Design review of the part built by this model. Coordinates are the model's own, in mm. Face numbers are marked on the shaded views. A direction names the side the tool comes from. Give positions to 0.01 mm unless a question says otherwise; leave off trailing zeros. Loops run counter-clockwise (first coordinate to the right, second up) from the corner with the lowest first, then second, coordinate; pieces in that order, holes last. Notation, with made-up numbers: M 21.5,76.5 L 52.5,76.5 A15 ccw 52.5,99.5 Z; hole C -24,-21.5 d1. An arc over 180 degrees is marked long. Use CSV: the item, a comma, the result in double quotes.
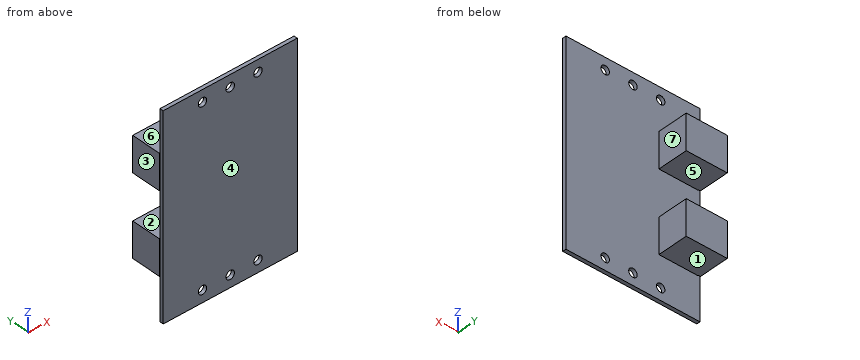
from build123d import *

# Parameters (mm, degrees)
SKETCH_1_W          = 60.4
SKETCH_1_H          = 89.7
EXTRUDE_1_DEPTH     = 1.6
SKETCH_2_R          = 1.9
CUT_EXTRUDE_1_DEPTH = 1.6
SKETCH_3_W          = 15.8
SKETCH_3_H          = 13.7
EXTRUDE_2_DEPTH     = 18.5
SKETCH_4_W          = 51.8
SKETCH_4_H          = 0.2
CUT_EXTRUDE_2_DEPTH = 1


with BuildPart() as part:
    # 草图1 → 凸台-拉伸1 (new body)
    with BuildSketch(Plane(origin=(0, 0, 0), x_dir=(1, 0, 0), z_dir=(0, 1, 0))):
        Rectangle(SKETCH_1_W, SKETCH_1_H)
    extrude(amount=EXTRUDE_1_DEPTH)

    # 草图2 → 切除-拉伸1 (cut)
    with BuildSketch(Plane(origin=(0, 1.6, 0), x_dir=(1, 0, 0), z_dir=(0, 1, 0))):
        with Locations(Location((-12.5, -39.5, 0), (0, 0, 270))):
            Circle(SKETCH_2_R)
        with Locations(Location((12.5, -39.5, 0), (0, 0, 270))):
            Circle(SKETCH_2_R)
        with Locations(Location((-12.5, 39.5, 0), (0, 0, 270))):
            Circle(SKETCH_2_R)
        with Locations(Location((12.5, 39.5, 0), (0, 0, 270))):
            Circle(SKETCH_2_R)
        with Locations(Location((0, 39.5, 0), (0, 0, 270))):
            Circle(SKETCH_2_R)
        with Locations(Location((0, -39.5, 0), (0, 0, 270))):
            Circle(SKETCH_2_R)
    extrude(amount=-CUT_EXTRUDE_1_DEPTH, mode=Mode.SUBTRACT)

    # 草图3 → 凸台-拉伸2 (add)
    with BuildSketch(Plane.ZY.offset(30.2)):
        with Locations((18, 8.45)):
            Rectangle(SKETCH_3_W, SKETCH_3_H)
        with Locations((-18, 8.45)):
            Rectangle(SKETCH_3_W, SKETCH_3_H)
    extrude(amount=-EXTRUDE_2_DEPTH)

    # 草图4 → 切除-拉伸2 (cut)
    with BuildSketch(Plane.ZY.offset(30.2)):
        with Locations((0, 1.7)):
            Rectangle(SKETCH_4_W, SKETCH_4_H)
    extrude(amount=-CUT_EXTRUDE_2_DEPTH, mode=Mode.SUBTRACT)


solid = part.part
(1) We need section D-D on x = -22. State the section outline as (y, z) points, then the cut area to 3 significant figures.
A:
outline,"M 0,-44.85 L 1.6,-44.85 L 1.6,-25.9 L 15.3,-25.9 L 15.3,-10.1 L 1.6,-10.1 L 1.6,10.1 L 15.3,10.1 L 15.3,25.9 L 1.6,25.9 L 1.6,44.85 L 0,44.85 Z"
area,"576 mm²"
(2) We need section A-A on z = -39.5. State the section outline as (x, y) points.
A:
outline,"M -30.2,0 L -14.4,0 L -14.4,1.6 L -30.2,1.6 Z; M -10.6,0 L -1.9,0 L -1.9,1.6 L -10.6,1.6 Z; M 1.9,0 L 10.6,0 L 10.6,1.6 L 1.9,1.6 Z; M 14.4,0 L 30.2,0 L 30.2,1.6 L 14.4,1.6 Z"
(3) Machinability: for the marked faces 4, 5, 6 and 7, which of the approach directions +Z, -Z, +X, -X, +Y, -Y give a long, thin tool a straight path to every point of the face, cutting with its end or side? Answer none if there is none.
A:
face 4,"+Z, -Z, +X, -X, -Y"
face 5,"+X, -X, +Y"
face 6,"+Z, +X, -X, +Y"
face 7,"+Z, -Z, +X, +Y"
(4) The part is to be moulded in two halves that separate along Z. For the marked faces 1, 2 and 3, say which applies: released by +Z, released by -Z, zero draft, split by the parting line, or undercut.
A:
face 1,"released by -Z"
face 2,"undercut"
face 3,"zero draft"
(5) Wall thickness on line 1 along X through (y, z) = (0.4, -39.5); line 2 along Z through (x, y) = (-17, 3.5); line 3 along Y through (x, z) = (-26, 34): over which ranges is each line inside the solid? List them lowest first. Write a range as [from, to].
A:
line 1,"[-30.2, -14.4], [-10.6, -1.9], [1.9, 10.6], [14.4, 30.2]"
line 2,"[-25.9, -10.1], [10.1, 25.9]"
line 3,"[0, 1.6]"
(6) We need section B-B on x = 0. State the section outline as (y, z) points, then the cut area to 3 significant figures.
A:
outline,"M 0,-44.85 L 1.6,-44.85 L 1.6,-41.4 L 0,-41.4 Z; M 0,-37.6 L 1.6,-37.6 L 1.6,37.6 L 0,37.6 Z; M 0,41.4 L 1.6,41.4 L 1.6,44.85 L 0,44.85 Z"
area,"131 mm²"
(7) We need section C-C on y = 11. State the section outline as (x, z) points.
A:
outline,"M -30.2,-25.9 L -11.7,-25.9 L -11.7,-10.1 L -30.2,-10.1 Z; M -30.2,10.1 L -11.7,10.1 L -11.7,25.9 L -30.2,25.9 Z"
(8) Clearance check with flat-ended pins moving along their axes: P1, Ø3.5, axis at x = 12.5, z = -39.5, coming from the -Y side; P2, Ø5, axis at y = 3.5, z = -27, coming from the -X side; P3, Ø4.5, axis at x = 0, z = 39.5, coming from the +Y side. State where each tip first meets the part, or that it passes through.
A:
P1,"through"
P2,"x = -30.2"
P3,"y = 1.6"
